```python
from build123d import *

# Parameters (mm, degrees)
SKETCH1_R             = 42.5
SKETCH1_R_2           = 25
BOSS_EXTRUDE1_DEPTH   = 8
SKETCH2_R             = 30
SKETCH2_R_2           = 25
BOSS_EXTRUDE2_DEPTH   = 3
CHAMFER1_SIZE         = 1
M4_TAPPED_HOLE1_D     = 3.3
M4_TAPPED_HOLE1_DEPTH = 6
M4_TAPPED_HOLE1_TIP   = 0.991420021


with BuildPart() as part:
    # Sketch1 → Boss-Extrude1 (new body)
    with BuildSketch(Plane.XY):
        Circle(SKETCH1_R)
        Circle(SKETCH1_R_2, mode=Mode.SUBTRACT)
    extrude(amount=BOSS_EXTRUDE1_DEPTH)

    # Sketch2 → Boss-Extrude2 (add)
    with BuildSketch(Plane.XY.offset(8)):
        Circle(SKETCH2_R)
        Circle(SKETCH2_R_2, mode=Mode.SUBTRACT)
    extrude(amount=BOSS_EXTRUDE2_DEPTH)

    # Chamfer1
    chamfer1_edges = [part.edges().sort_by_distance(p)[0] for p in [
        (-30, 0, 11),
        (-25, 0, 0),
    ]]
    chamfer(chamfer1_edges, length=CHAMFER1_SIZE)

    # M4 Tapped Hole1
    with Locations(Plane(origin=(18.5, 32.04293994, 0), x_dir=(-1, 0, 0), z_dir=(0, 0, -1))):
        with Locations((0, 0), (37, 0), (55.5, -32.04293994), (37, -64.08587988), (0, -64.08587988), (-18.5, -32.04293994)):
            Hole(M4_TAPPED_HOLE1_D / 2, depth=M4_TAPPED_HOLE1_DEPTH)
            with Locations((0, 0, -(M4_TAPPED_HOLE1_DEPTH + M4_TAPPED_HOLE1_TIP / 2))):  # 118° drill point
                Cone(0, M4_TAPPED_HOLE1_D / 2, M4_TAPPED_HOLE1_TIP, mode=Mode.SUBTRACT)


solid = part.part
```
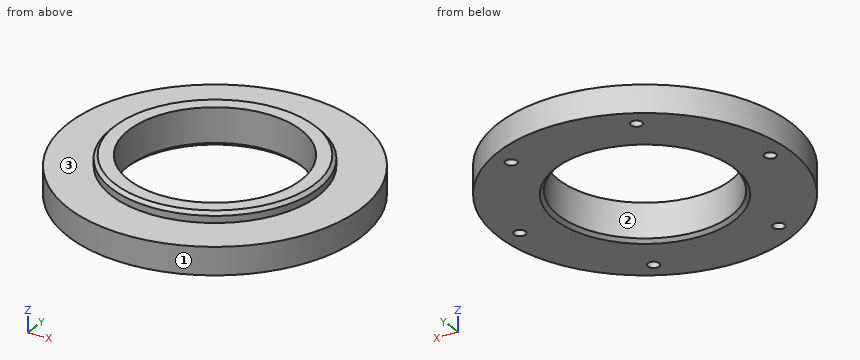
Check sheet for the modelled part. Datum: model origin and axes. Units: mm. Face numbers are marked on the shaded views. Round coordinates to 2 decimals unless told otherwise and drop trailing zeros. Order: outer loops, then holes, each group sorted by start corner. A loop starts at its lowest first (then second) coordinate and runs counter-clockwise, first axis right, second up.
1) Scan lines: line 1 (Y direction, x = 18.5, z = 1.4); line 2 (Y direction, x = 0, z = 8.75); line 3 (Z direction, x = 28, y = 24). Record each from-to range of solid material in increasing order.
2) Go/stop test with flat-tipped pins: pin 1 Ø1 at (x, z) = (8, 2) entering from -Y; pin 2 Ø1.5 at (x, z) = (21.5, 9) entering from -Y; pin 3 Ø2 at (x, z) = (10.5, 2.5) entering from +Y; pin 4 Ø1 at (x, y) = (2.5, 23.5) entering from -Z. Record where each tip stops, or that it passes through.
3) Mould release check, pull along X, two halves, no side actions. Record for the marked faces 1, 2 and 3: +X half, -X half, draft (parallel to the pull), parting line (faces both ways), or undercut.
4) Section check B-B (x = 31). Record the boundary of the cut face in (y, z), and give its area (3 significant figures).
5) Section check A-A (z = 3.25). Record the boundary of the cut face in (x, y).
Result:
1. line 1: y = -38.26 to -33.69, -30.39 to -16.82, 16.82 to 30.39, 33.69 to 38.26
1. line 2: y = -30 to -25, 25 to 30
1. line 3: z = 0 to 8
2. pin 1: stops at y = -41.83
2. pin 2: stops at y = -21.67
2. pin 3: stops at y = 41.42
2. pin 4: passes through
3. face 1: parting line
3. face 2: undercut
3. face 3: draft
4. outline: (-29.07, 0) - (29.07, 0) - (29.07, 8) - (-29.07, 8) - close
4. area: 465 mm2
5. outline: circle Ø85 at (0, 0); hole circle Ø3.3 at (-37, 0); hole circle Ø50 at (0, 0); hole circle Ø3.3 at (-18.5, -32.04); hole circle Ø3.3 at (-18.5, 32.04); hole circle Ø3.3 at (18.5, -32.04); hole circle Ø3.3 at (18.5, 32.04); hole circle Ø3.3 at (37, 0)
